Verification items for the finished model (mm, model axes). A direction names the side the tool comes from. Give positions to 0.01 mm unless a question says otherwise; leave off trailing zeros. Order: outer loops, then holes, each group sorted by start corner. A loop starts at its lowest first (then second) coordinate and runs counter-clockwise, first axis right, second up. Notation, with made-up numbers: M 64,57 L 90,57 A6 ccw 90,61 Z; hole C 11,-19 d6. An arc over 180 degrees is marked long. Answer as a JSON object with one key per item and string values.
```python
from build123d import *

# Parameters (mm, degrees)
UNEQUAL_ANGLE_6_3_4_5_1_DEPTH = 50
SKETCH3_R                     = 8.5
CUT_EXTRUDE1_DEPTH            = 10


with BuildPart() as part:
    # Sketch1 → Unequal Angle 6.3-4-5(1) (new body)
    with BuildSketch(Plane(origin=(0, 0, 0), x_dir=(0, 0, 1), z_dir=(1, 0, 0))):
        with BuildLine():
            Line((63, 0), (0, 0))
            Line((0, 0), (0, -40))
            Line((0, -40), (3.333333333, -40))
            ThreePointArc((3.333333333, -40), (4.511844635, -39.511844635), (5, -38.333333333))
            Line((5, -38.333333333), (5, -12))
            ThreePointArc((5, -12), (7.050252532, -7.050252532), (12, -5))
            Line((12, -5), (61.333333333, -5))
            ThreePointArc((61.333333333, -5), (62.511844635, -4.511844635), (63, -3.333333333))
            Line((63, -3.333333333), (63, 0))
        make_face()
    extrude(amount=UNEQUAL_ANGLE_6_3_4_5_1_DEPTH)

    # Sketch3 → Cut-Extrude1 (cut)
    with BuildSketch(Plane(origin=(0, 5, 0), x_dir=(1, 0, 0), z_dir=(0, 1, 0))):
        with Locations(Location((25, -43, 0), (0, 0, 270))):
            Circle(SKETCH3_R)
    extrude(amount=-CUT_EXTRUDE1_DEPTH, mode=Mode.SUBTRACT)


solid = part.part
```
Q1. Section check D-D on y = 24.5. Record the cut outline in (x, z), then the cut area to 3 significant figures.
Resolved:
{"outline": "M 0,0 L 50,0 L 50,5 L 0,5 Z", "area": "250 mm²"}
Q2. Gauge pin test, flat ends, axial feed: pin 1 Ø8 at (x, y) = (11, 8) entering from +Z; pin 2 Ø2 at (x, y) = (41, 29) entering from +Z; pin 3 Ø24.5 at (x, z) = (37, 40) entering from +Y. Record the tip position at first contact, or that the pin passes through.
Resolved:
{"pin 1": "stops at z = 62.86", "pin 2": "stops at z = 5", "pin 3": "stops at y = 5"}
Q3. Section check A-A on z = 43. Record the cut outline in (x, y).
Resolved:
{"outline": "M 0,0 L 16.5,0 L 16.5,5 L 0,5 Z; M 33.5,0 L 50,0 L 50,5 L 33.5,5 Z"}
Q4. Tool access check on faces 1 (the face through (25, 5, 31)), 2 (the face through (25, 0, 32)). Record the directions out of +Z, -Z, +X, -X, +Y, -Y that give a thin tool (end or side, any length) a straight path to the whole face; none if there is none.
Resolved:
{"face 1": "+Z, +X, -X, +Y", "face 2": "+Z, -Z, +X, -X, -Y"}
Q5. Section check B-B on x = 21. Record the cut outline in (y, z).
Resolved:
{"outline": "M 0,0 L 40,0 L 40,3.33 A1.67 ccw 38.33,5 L 12,5 A7 cw 5,12 L 5,35.5 L 0,35.5 Z; M 0,50.5 L 5,50.5 L 5,61.33 A1.67 ccw 3.33,63 L 0,63 Z"}
Q6. Section check C-C on x = 8. Record the cut outline in (y, z).
Resolved:
{"outline": "M 0,0 L 40,0 L 40,3.33 A1.67 ccw 38.33,5 L 12,5 A7 cw 5,12 L 5,61.33 A1.67 ccw 3.33,63 L 0,63 Z"}
Q7. Release check for a two-part mould opening along X. For faces 3 (the face through (50, 4, 20)), 4 (the face through (19.828, 2.535, 36.255)), 5 (the face through (24.6, 7.1, 7)) record: +X half, -X half, draft (parallel to the pull), parting line (faces both ways), or undercut.
Resolved:
{"face 3": "+X half", "face 4": "undercut", "face 5": "draft"}
Q8. Material ranges on L1, parallel to X at y = 1, z = 43; L2, parallel to Y at x = 21.5, z = 21, recorded low to high.
Resolved:
{"L1": "x = 0 to 16.5, 33.5 to 50", "L2": "y = 0 to 5"}
